CAD build for the part. Positions are in the model's coordinates, mm. A direction names the side the tool comes from. Give positions to 0.01 mm unless a question says otherwise; leave off trailing zeros. Write each loop counter-clockwise with the first axis right and the second up, starting at its lowest first coordinate (ties: lowest second). Pieces come first, ordered by that corner, then holes. Notation, with made-up numbers: (-23.5, 40) -> (11.5, 40) arc R28 ccw to (11.5, 59) -> close; hole circle Ø4 at (-20.5, 70). An arc over 180 degrees is marked (long way). Answer as a JSON object with one key per item and string values.
```python
from build123d import *

# Parameters (mm, degrees)
SKETCH1_R           = 15
BOSS_EXTRUDE1_DEPTH = 150
SKETCH3_W           = 13.5
SKETCH3_H           = 147.5
SKETCH3_H_2         = 0.5
CHAMFER1_SIZE       = 0.5


with BuildPart() as part:
    # Sketch1 → Boss-Extrude1 (new body)
    with BuildSketch(Plane(origin=(0, 0, 0), x_dir=(1, 0, 0), z_dir=(0, 1, 0))):
        with Locations(Location((0, 0, 0), (0, 0, 270))):
            Circle(SKETCH1_R)
    extrude(amount=BOSS_EXTRUDE1_DEPTH)

    # Sketch3 → Cut-Revolve1 (revolve, cut)
    with BuildSketch(Plane.XY, mode=Mode.PRIVATE) as cut_revolve1_sk:
        with Locations((6.75, 76.25)):
            Rectangle(SKETCH3_W, SKETCH3_H)
        with Locations((6.75, 0.25)):
            Rectangle(SKETCH3_W, SKETCH3_H_2)
    revolve(cut_revolve1_sk.sketch.rotate(Axis((0, 0, 0), (0, 1, 0)), 90), axis=Axis((0, 0, 0), (0, 1, 0)), mode=Mode.SUBTRACT)

    # Chamfer1
    chamfer1_edges = [part.edges().sort_by_distance(p)[0] for p in [
        (0, 0, -15),
    ]]
    chamfer(chamfer1_edges, length=CHAMFER1_SIZE)


solid = part.part
```
1) Slice it at B-B (x = 0). List the corners of the cut face in (y, z), then the cut area to 3 significant figures.
Model answer:
{"outline": "(0, -14.5) -> (0.5, -15) -> (150, -15) -> (150, -13.5) -> (2.5, -13.5) -> (2.5, 13.5) -> (150, 13.5) -> (150, 15) -> (0.5, 15) -> (0, 14.5) -> (0, 13.5) -> (0.5, 13.5) -> (0.5, -13.5) -> (0, -13.5) -> close", "area": "504 mm2"}
2) Pin check, flat tips, straight feed: pin 1 (8 mm diameter, centred on x = -4.5, z = -2, fed in from +Y); pin 2 (1 mm diameter, centred on y = 99, z = -3.5, fed in from +X); pin 3 (2 mm diameter, centred on x = -6, z = -4.5, fed in from -Y). Stop position of each tip, or through.
Model answer:
{"pin 1": "stops at y = 2.5", "pin 2": "stops at x = 14.7", "pin 3": "stops at y = 0.5"}
3) Slice it at A-A (z = 0). List the corners of the cut face in (x, y), then the cut area to 3 significant figures.
Model answer:
{"outline": "(-15, 0.5) -> (-14.5, 0) -> (-13.5, 0) -> (-13.5, 0.5) -> (13.5, 0.5) -> (13.5, 0) -> (14.5, 0) -> (15, 0.5) -> (15, 150) -> (13.5, 150) -> (13.5, 2.5) -> (-13.5, 2.5) -> (-13.5, 150) -> (-15, 150) -> close", "area": "504 mm2"}
4) Mould opens along Z. For faces 4 (the flat face through (0, 2.5, 0)), 5 (the flat face through (7.85, 150, -11.18)), 6 (the cylindrical face through (0.66, 74.204, -14.985)) say: released by +Z, released by -Z, zero draft, split by the parting line, or undercut.
Model answer:
{"face 4": "undercut", "face 5": "zero draft", "face 6": "split by the parting line"}
5) 3-axis set-ups, long thin cutter, end or side, ignore diameter. For faces 1 (the cylindrical face through (13.18, 0.25, 2.93)), 2 (the flat face through (-10, 0, 10)), 3 (the cylindrical face through (13.18, 77.28, 2.93)): which of +Z, -Z, +X, -X, +Y, -Y reach the whole face in a straight line?
Model answer:
{"face 1": "-Y", "face 2": "+Z, -Z, +X, -X, -Y", "face 3": "+Y"}
6) Wall check: probe 1 along Z at (x, y) = (0.5, 35); probe 2 along Z at (x, y) = (-9, 119). Give the ranges that are in metal, low to high.
Model answer:
{"probe 1": "z = -14.99 to -13.49, 13.49 to 14.99", "probe 2": "z = -12 to -10.06, 10.06 to 12"}
7) Slice it at C-C (y = 88). List the corners of the cut face in (x, z).
Model answer:
{"outline": "circle Ø30 at (0, 0); hole circle Ø27 at (0, 0)"}
